Geometry check sheet. Reference: the model listing, model coordinates, mm. A direction names the side the tool comes from. Round coordinates to 2 decimals unless told otherwise and drop trailing zeros. Loops run counter-clockwise (first coordinate to the right, second up) from the corner with the lowest first, then second, coordinate; pieces in that order, holes last.
```python
from build123d import *

# Parameters (mm, degrees)
CHAMFER_1_SIZE = 5


with BuildPart() as part:
    # 草图2 → 旋转1 (revolve)
    with BuildSketch(Plane.XY, mode=Mode.PRIVATE) as revolve_1_sk:
        Polygon((-35, 33), (-39.5, 33), (-39.5, 27), (-47.5, 27), (-47.5, 0), (-42.5, 0), (-42.5, 18), (-35, 18), align=None)
    revolve(revolve_1_sk.sketch.rotate(Axis((0, 0, 0), (0, 1, 0)), 270), axis=Axis((0, 0, 0), (0, 1, 0)))

    # 倒角1
    chamfer_1_edges = [part.edges().sort_by_distance(p)[0] for p in [
        (0, 18, 35),
    ]]
    chamfer(chamfer_1_edges, length=CHAMFER_1_SIZE)


solid = part.part
```
1) Sectioned sample at C-C, the plane y = 14. Record the cut outline in (x, z), then the cut area to 3 significant figures.
Report:
outline: circle Ø95 at (0, 0); hole circle Ø85 at (0, 0)
area: 1,410 mm2
2) Sectioned sample at A-A, the plane z = 0. Record the cut outline in (x, y), then the cut area to 3 significant figures.
Report:
outline: (-47.5, 0) - (-42.5, 0) - (-42.5, 18) - (-40, 18) - (-35, 23) - (-35, 33) - (-39.5, 33) - (-39.5, 27) - (-47.5, 27) - close; (35, 23) - (40, 18) - (42.5, 18) - (42.5, 0) - (47.5, 0) - (47.5, 27) - (39.5, 27) - (39.5, 33) - (35, 33) - close
area: 434 mm2
3) Gauge pin test, flat ends, axial feed: pin 1 (10 mm diameter, centred on x = -14, y = 25, fed in from +Z); pin 2 (3 mm diameter, centred on y = 21.5, z = -22.5, fed in from +X); pin 3 (6 mm diameter, centred on x = -36.5, z = -9.5, fed in from -Y). Record the tip position at first contact, or that the pin passes through.
Report:
pin 1: stops at z = 46.64
pin 2: stops at x = 42.61
pin 3: stops at y = 18
4) Sectioned sample at B-B, the plane x = 0. Record the cut outline in (y, z).
Report:
outline: (0, -47.5) - (27, -47.5) - (27, -39.5) - (33, -39.5) - (33, -35) - (23, -35) - (18, -40) - (18, -42.5) - (0, -42.5) - close; (0, 42.5) - (18, 42.5) - (18, 40) - (23, 35) - (33, 35) - (33, 39.5) - (27, 39.5) - (27, 47.5) - (0, 47.5) - close
5) Mould release check, pull along X, two halves, no side actions. Record for faces 4 (the face through (25.861, 9.126, 33.727)), 5 (the face through (-11.865, 29.958, -37.676)), 6 (the face through (24.4, 0, 35.4)): +X half, -X half, draft (parallel to the pull), parting line (faces both ways), or undercut.
Report:
face 4: undercut
face 5: parting line
face 6: draft
6) Sectioned sample at D-D, the plane y = 29. Record the cut outline in (x, z).
Report:
outline: circle Ø79 at (0, 0); hole circle Ø70 at (0, 0)
7) Scan lines: line 1 along X through (y, z) = (11, 0); line 2 along X through (y, z) = (29, 0); line 3 along Z through (x, y) = (-26, 26.5). Record each from-to range of solid material in increasing order.
Report:
line 1: x = -47.5 to -42.5, 42.5 to 47.5
line 2: x = -39.5 to -35, 35 to 39.5
line 3: z = -39.75 to -23.43, 23.43 to 39.75
8) Access from +Z, -Z, +X, -X, +Y, -Y to the whole of each face (thin tool, end or side, straight path). Record for faces 1 (the face through (46.37, 13.31, 10.3)), 2 (the face through (28, 18, 29)), 3 (the face through (10, 27, -39)).
Report:
face 1: +Y, -Y
face 2: -Y
face 3: +Y
